Check sheet for the modelled part. Datum: model origin and axes. Units: mm. A direction names the side the tool comes from. Round coordinates to 2 decimals unless told otherwise and drop trailing zeros. Order: outer loops, then holes, each group sorted by start corner. A loop starts at its lowest first (then second) coordinate and runs counter-clockwise, first axis right, second up. Notation, with made-up numbers: (-9, 24) -> (39, 24) arc R26 ccw to (39, 40) -> close; hole circle Ø4 at (-23.75, 65.25). An arc over 180 degrees is marked (long way). Answer in a Markdown table with one row per item. Add a question column.
1. Sectioned sample at B-B, the plane y = -35. Record the boundary of the cut face in (x, z).
2. Access from +Z, -Z, +X, -X, +Y, -Y to the whole of each face (thin tool, end or side, straight path). Record for faces 4 (the flat face through (-1, 55, 0)), 5 (the flat face through (-30.2, -10, 0)).
3. Sectioned sample at D-D, the plane y = 47. Record the boundary of the cut face in (x, z).
4. Sectioned sample at A-A, the plane x = 0. Record the boundary of the cut face in (y, z), then the cut area to 3 significant figures.
5. Draft check along X on faces 1 (the flat face through (70, -1, 0)), 2 (the flat face through (-1, -55, 0)), 3 (the cylindrical face through (46.34, -33.48, -0.02)). Enter one of: +X half, -X half, draft (parallel to the pull), parting line (faces both ways), or undercut.
6. Material ranges on L1, parallel to Y at x = 0, z = 0.9; L2, parallel to Y at x = 42, z = 0.45; L3, parallel to Y at x = -26.5, z = 0.85, recorded low to high. Write a range as from..to.
7. Sectioned sample at C-C, the plane x = -28.5. Record the boundary of the cut face in (y, z).
```python
from build123d import *

# Parameters (mm, degrees)
SKETCH_1_W      = 140
SKETCH_1_H      = 110
SKETCH_1_R      = 2.25
SKETCH_1_R_2    = 6.1
SKETCH_1_R_3    = 8.1
SKETCH_1_R_4    = 4.6
SKETCH_1_W_2    = 60.4
SKETCH_1_H_2    = 34.4
EXTRUDE_1_DEPTH = 1.5


with BuildPart() as part:
    # 草图1 → 凸台-拉伸1 (new, symmetric)
    with BuildSketch(Plane.XY):
        Rectangle(SKETCH_1_W, SKETCH_1_H)
        with Locations((-62, -47)):
            Circle(SKETCH_1_R, mode=Mode.SUBTRACT)
        with Locations((-62, 47)):
            Circle(SKETCH_1_R, mode=Mode.SUBTRACT)
        with Locations((62, -47)):
            Circle(SKETCH_1_R, mode=Mode.SUBTRACT)
        with Locations((62, 47)):
            Circle(SKETCH_1_R, mode=Mode.SUBTRACT)
        with Locations((-42, 30)):
            Circle(SKETCH_1_R_2, mode=Mode.SUBTRACT)
        with Locations((42, 30)):
            Circle(SKETCH_1_R_3, mode=Mode.SUBTRACT)
        with Locations((0, 38)):
            Circle(SKETCH_1_R_4, mode=Mode.SUBTRACT)
        with Locations((48, -35)):
            Circle(SKETCH_1_R, mode=Mode.SUBTRACT)
        with Locations((0, -10)):
            Rectangle(SKETCH_1_W_2, SKETCH_1_H_2, mode=Mode.SUBTRACT)
    extrude(amount=EXTRUDE_1_DEPTH, both=True)


solid = part.part
```
Answer key:
| question | item | result |
|---|---|---|
| 1 | outline | (-70, -1.5) -> (45.75, -1.5) -> (45.75, 1.5) -> (-70, 1.5) -> close; (50.25, -1.5) -> (70, -1.5) -> (70, 1.5) -> (50.25, 1.5) -> close |
| 2 | face 4 | +Z, -Z, +X, -X, +Y |
| 2 | face 5 | +Z, -Z |
| 3 | outline | (-70, -1.5) -> (-64.25, -1.5) -> (-64.25, 1.5) -> (-70, 1.5) -> close; (-59.75, -1.5) -> (59.75, -1.5) -> (59.75, 1.5) -> (-59.75, 1.5) -> close; (64.25, -1.5) -> (70, -1.5) -> (70, 1.5) -> (64.25, 1.5) -> close |
| 4 | outline | (-55, -1.5) -> (-27.2, -1.5) -> (-27.2, 1.5) -> (-55, 1.5) -> close; (7.2, -1.5) -> (33.4, -1.5) -> (33.4, 1.5) -> (7.2, 1.5) -> close; (42.6, -1.5) -> (55, -1.5) -> (55, 1.5) -> (42.6, 1.5) -> close |
| 4 | area | 199 mm² |
| 5 | face 1 | +X half |
| 5 | face 2 | draft |
| 5 | face 3 | undercut |
| 6 | L1 | y = -55..-27.2, 7.2..33.4, 42.6..55 |
| 6 | L2 | y = -55..21.9, 38.1..55 |
| 6 | L3 | y = -55..-27.2, 7.2..55 |
| 7 | outline | (-55, -1.5) -> (-27.2, -1.5) -> (-27.2, 1.5) -> (-55, 1.5) -> close; (7.2, -1.5) -> (55, -1.5) -> (55, 1.5) -> (7.2, 1.5) -> close |
